Verification items for this drawing (mm, ordinates from the low corner). Round coordinates to 2 decimals unless told otherwise and drop trailing zeros. Order: outer loops, then holes, each group sorted by start corner. A loop starts at its lowest first (then second) coordinate and runs counter-clockwise, first axis right, second up. Notation, with made-up numbers: (57.5, -33.5) - (106.5, -33.5) arc R28 cw to (106.5, -11.5) - close; hole circle Ø2 at (26.5, -37.5). An arc over 180 degrees is marked (long way). Return JSON: item names as keys, results as strings. Group by question number.
Q1. Draft check along X on the marked faces 1, 2 and 3. Enter one of: pulls with the +X half, pulls with the -X half, needs draft (parallel to the pull), parting line crosses it, or undercut.
Q2. Gauge pin test, flat end, axial feed: pin 1 Ø7.5 at (y, z) = (70, 102) entering from -X. Record the tip position at first contact, or that the pin passes through.
Q3. Sectioned sample at D-D, the plane x = 3.75. Record the cut outline in (y, z).
Q4. Sectioned sample at B-B, the plane z = 101. Record the cut outline in (x, y), then the cut area to 3 significant figures.
Q5. Sectioned sample at A-A, the plane z = 9. Record the cut outline in (x, y).
Q6. Material ranges on line 1 along Y through (x, z) = (4.75, 27); line 2 along Z through (x, y) = (9.25, 13); line 3 along Y through (x, z) = (9.7, 27), recorded low to high.
Q7. Sectioned sample at C-C, the plane y = 67.5. Record the cut outline in (x, z), then the cut area to 3 significant figures.
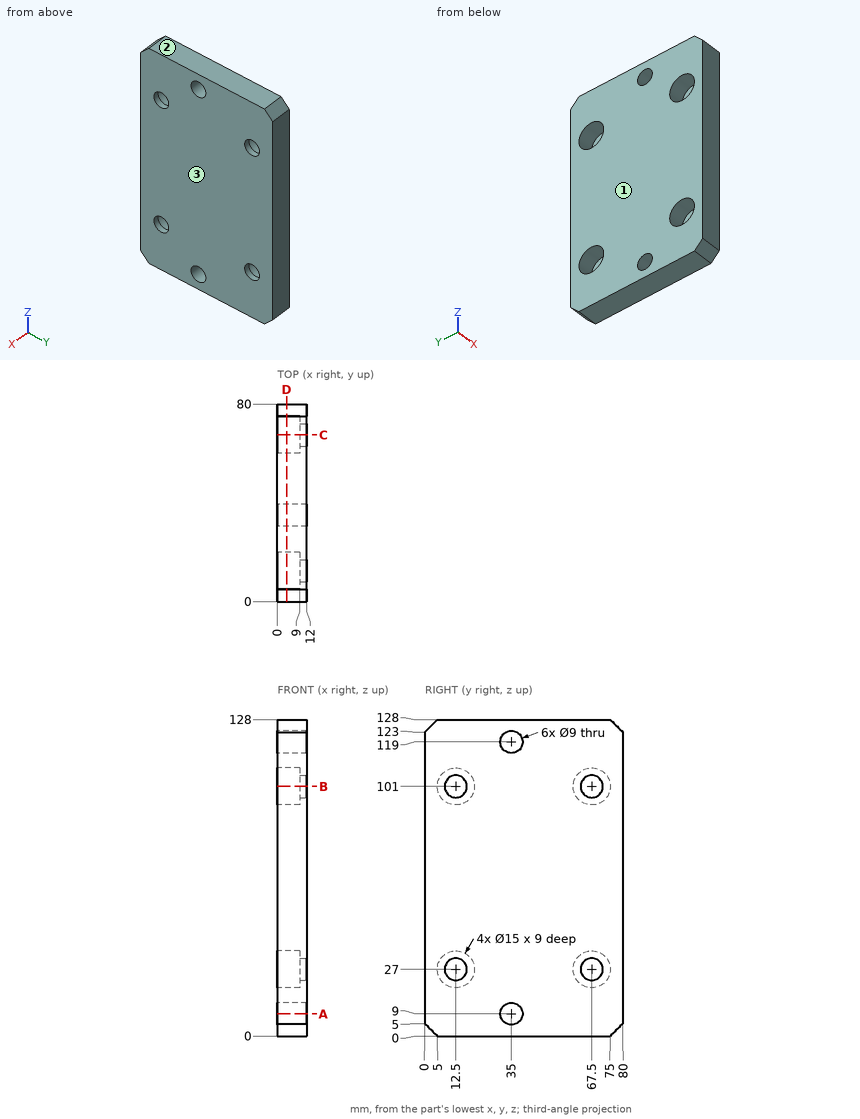
Reply:
{
 "1": {"face 1": "pulls with the -X half", "face 2": "needs draft", "face 3": "pulls with the +X half"},
 "2": {"pin 1": "x = 9"},
 "3": {"outline": "(0, 5) - (5, 0) - (75, 0) - (80, 5) - (80, 123) - (75, 128) - (5, 128) - (0, 123) - close; hole circle Ø15 at (12.5, 27); hole circle Ø15 at (12.5, 101); hole circle Ø9 at (35, 9); hole circle Ø9 at (35, 119); hole circle Ø15 at (67.5, 27); hole circle Ø15 at (67.5, 101)"},
 "4": {"outline": "(0, 0) - (12, 0) - (12, 8) - (9, 8) - (9, 5) - (0, 5) - close; (0, 20) - (9, 20) - (9, 17) - (12, 17) - (12, 63) - (9, 63) - (9, 60) - (0, 60) - close; (0, 75) - (9, 75) - (9, 72) - (12, 72) - (12, 80) - (0, 80) - close", "area": "636 mm^2"},
 "5": {"outline": "(0, 0) - (12, 0) - (12, 30.5) - (0, 30.5) - close; (0, 39.5) - (12, 39.5) - (12, 80) - (0, 80) - close"},
 "6": {"line 1": "0 to 5, 20 to 60, 75 to 80", "line 2": "0 to 22.53, 31.47 to 96.53, 105.47 to 128", "line 3": "0 to 8, 17 to 63, 72 to 80"},
 "7": {"outline": "(0, 0) - (12, 0) - (12, 22.5) - (9, 22.5) - (9, 19.5) - (0, 19.5) - close; (0, 34.5) - (9, 34.5) - (9, 31.5) - (12, 31.5) - (12, 96.5) - (9, 96.5) - (9, 93.5) - (0, 93.5) - close; (0, 108.5) - (9, 108.5) - (9, 105.5) - (12, 105.5) - (12, 128) - (0, 128) - close", "area": "1,210 mm^2"}
}
